Read the model definition and answer for the solid it produces. Units are mm, in the model's axes. Face numbers are marked on the shaded views. A direction names the side the tool comes from. Give positions to 0.01 mm unless a question says otherwise; leave off trailing zeros. Write each loop counter-clockwise with the first axis right and the second up, starting at its lowest first coordinate (ties: lowest second). Pieces come first, ordered by that corner, then holes.
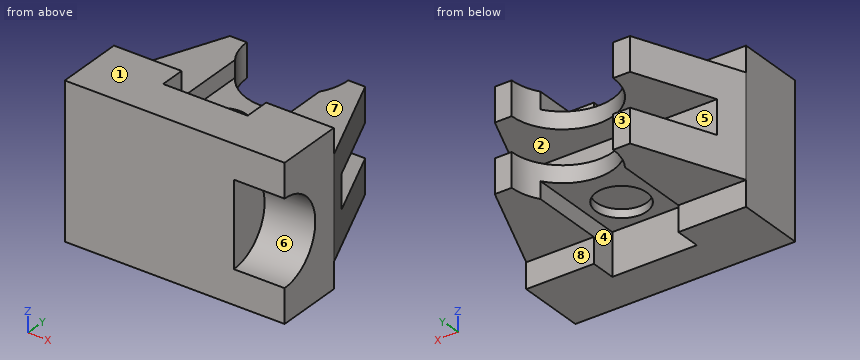
```python
from build123d import *

# Parameters (mm, degrees)
BASE_BLOCK_DEPTH        = 45
BOTTOM_ARCH_CUT_DEPTH   = 30
BEARING_PEDESTAL_DEPTH  = 75
PEDESTAL_SIDE_CUT_DEPTH = 15
BEARING_SEAT_PROFILE_W  = 130
BEARING_SEAT_PROFILE_H  = 20
BEARING_SEAT_CUT_DEPTH  = 45
CROSS_HOLE_DEPTH        = 114.468057179
CROSS_HOLE_DEPTH_BACK   = 114.468057179
SLOT_A_CUT_DEPTH        = 10
SLOT_START              = -10
SLOT_B_CUT_DEPTH        = 10
STEP_RECESS_A_PROFILE_R = 15
STEP_RECESS_A_DEPTH     = 5
STEP_RECESS_B_PROFILE_R = 15
STEP_RECESS_B_DEPTH     = 5


with BuildPart() as part:
    # Base Block Profile → Base Block (new, symmetric)
    with BuildSketch(Plane.XY):
        Polygon((0, 0), (25, 0), (25, 15), (65, 15), (65, -25), (-65, -25), (-65, 15), (-25, 15), (-25, 0), align=None)
    extrude(amount=BASE_BLOCK_DEPTH, both=True)

    # Bottom Arch Profile R25 → Bottom Arch Cut (cut)
    with BuildSketch(Plane(origin=(65, 0, 0), x_dir=(0, 0, -1), z_dir=(1, 0, 0))):
        with BuildLine():
            Line((-25, -25), (25, -25))
            ThreePointArc((25, -25), (0, 0), (-25, -25))
        make_face()
    extrude(amount=-BOTTOM_ARCH_CUT_DEPTH, mode=Mode.SUBTRACT)

    # Pedestal Profile → Bearing Pedestal (add)
    with BuildSketch(Plane.XY.offset(45)):
        Polygon((-65, 15), (-40, 75), (40, 75), (65, 15), (25, 15), (25, 0), (-25, 0), (-25, 15), align=None)
    extrude(amount=-BEARING_PEDESTAL_DEPTH)

    # Pedestal Side Cut Profile → Pedestal Side Cut (cut)
    with BuildSketch(Plane.XY.offset(45)):
        Polygon((-65, 15), (-25, 15), (-25, 0), (25, 0), (25, 15), (65, 15), (40, 75), (-40, 75), align=None)
    extrude(amount=-PEDESTAL_SIDE_CUT_DEPTH, mode=Mode.SUBTRACT)

    # Bearing Seat Profile → Bearing Seat Cut (cut)
    with BuildSketch(Plane(origin=(0, 75, 0), x_dir=(1, 0, 0), z_dir=(0, 1, 0))):
        Rectangle(BEARING_SEAT_PROFILE_W, BEARING_SEAT_PROFILE_H)
    extrude(amount=-BEARING_SEAT_CUT_DEPTH, mode=Mode.SUBTRACT)

    # Cross Hole Profile → Cross Hole (cut, two sides: drawn at the far end of the back side and taken through both)
    with BuildSketch(Plane(origin=(0, 0, 10), x_dir=(-1, 0, 0), z_dir=(0, 0, -1)).offset(-CROSS_HOLE_DEPTH_BACK)):
        with BuildLine():
            Line((-30, 75), (30, 75))
            ThreePointArc((30, 75), (0, 45), (-30, 75))
        make_face()
    extrude(amount=CROSS_HOLE_DEPTH + CROSS_HOLE_DEPTH_BACK, mode=Mode.SUBTRACT)

    # Slot A Profile → Slot A Cut (cut)
    with BuildSketch(Plane.XY.offset(30)):
        with BuildLine():
            Line((-25, 0), (-25, 58.416876048))
            ThreePointArc((-25, 58.416876048), (0, 45), (25, 58.416876048))
            Line((25, 58.416876048), (25, 0))
            Line((25, 0), (-25, 0))
        make_face()
    extrude(amount=-SLOT_A_CUT_DEPTH, mode=Mode.SUBTRACT)

    # Slot B Profile → Slot B Cut (cut)
    with BuildSketch(Plane(origin=(0, 0, -30), x_dir=(-1, 0, 0), z_dir=(0, 0, -1)).offset(SLOT_START)):
        with BuildLine():
            Line((-25, 0), (25, 0))
            Line((25, 0), (25, 58.416876048))
            ThreePointArc((25, 58.416876048), (0, 45), (-25, 58.416876048))
            Line((-25, 58.416876048), (-25, 0))
        make_face()
    extrude(amount=SLOT_B_CUT_DEPTH, mode=Mode.SUBTRACT)

    # Step Recess A Profile → Step Recess A (cut)
    with BuildSketch(Plane(origin=(0, 0, -20), x_dir=(-1, 0, 0), z_dir=(0, 0, -1))):
        with Locations((-5, 20)):
            Circle(STEP_RECESS_A_PROFILE_R)
    extrude(amount=-STEP_RECESS_A_DEPTH, mode=Mode.SUBTRACT)

    # Step Recess B Profile → Step Recess B (cut)
    with BuildSketch(Plane.XY.offset(20)):
        with Locations((-5, 20)):
            Circle(STEP_RECESS_B_PROFILE_R)
    extrude(amount=-STEP_RECESS_B_DEPTH, mode=Mode.SUBTRACT)


solid = part.part
```
Item 1: Section D-D (y = 61) is taken. Write down the section's boundary in (x, z), and give its area (3 significant figures).
Result set:
outline: (-45.83, -30) - (-26.53, -30) - (-26.53, -10) - (-45.83, -10) - close; (-45.83, 10) - (-26.53, 10) - (-26.53, 30) - (-45.83, 30) - close; (26.53, -30) - (45.83, -30) - (45.83, -10) - (26.53, -10) - close; (26.53, 10) - (45.83, 10) - (45.83, 30) - (26.53, 30) - close
area: 1,540 mm2
Item 2: Each of these flat-tipped pins is pushed along its axis until it touches: pin 1 Ø8 at (x, y) = (-27, 47.5) entering from +Z; pin 2 Ø22.5 at (x, y) = (-22.5, 62.5) entering from -Z; pin 3 Ø15 at (x, y) = (2, 17) entering from +Z; pin 4 Ø8 at (x, z) = (41.5, -19.5) entering from +Y. Where does it stop, or does it pass through?
Result set:
pin 1: stops at z = 30
pin 2: stops at z = -30
pin 3: stops at z = 20
pin 4: stops at y = 75
Item 3: Which of the six approach directions +Z, -Z, +X, -X, +Y, -Y give full straight-line access (tool end or side, diameter ignored) to the marked faces 4, 5, 6, 7 and 8?
Result set:
face 4: -Z, +Y
face 5: +X, -X, +Y
face 6: +X, -Y
face 7: +Z, +X, -X, +Y
face 8: -Z, +X, -X, +Y
Item 4: Determine the mould class of the marked faces 1, 2 and 3 for opening direction Z: pulls with the +Z half, pulls with the -Z half, needs draft (parallel to the pull), parting line crosses it, or undercut.
Result set:
face 1: pulls with the +Z half
face 2: undercut
face 3: needs draft
Item 5: Section C-C (x = 53) is taken. Write down the section's boundary in (y, z), and give its area (3 significant figures).
Result set:
outline: (-25, -45) - (15, -45) - (15, -30) - (43.8, -30) - (43.8, -10) - (30, -10) - (30, 10) - (43.8, 10) - (43.8, 30) - (15, 30) - (15, 45) - (-25, 45) - (-25, 25) arc R25 cw to (-25, -25) - close
area: 4,070 mm2
Item 6: Find the intervals of material crossed by line 1 along Z through (x, y) = (10, 44); line 2 along X through (y, z) = (6.5, 25); line 3 along Z through (x, y) = (-38.5, 50.5), in increasing order.
Result set:
line 1: z = -20 to -10, 10 to 20
line 2: x = -65 to -25, 25 to 65
line 3: z = -30 to -10, 10 to 30
Item 7: Section B-B (y = 41) is taken. Write down the section's boundary in (x, z).
Result set:
outline: (-54.17, -30) - (-25, -30) - (-25, -20) - (25, -20) - (25, -30) - (54.17, -30) - (54.17, -10) - (-54.17, -10) - close; (-54.17, 10) - (54.17, 10) - (54.17, 30) - (25, 30) - (25, 20) - (-25, 20) - (-25, 30) - (-54.17, 30) - close
Item 8: Section A-A (z = 0) is taken. Write down the section's boundary in (x, y).
Result set:
outline: (-65, -25) - (35, -25) - (35, 0) - (65, 0) - (65, 15) - (58.75, 30) - (-58.75, 30) - (-65, 15) - close
